Design review of the part built by this model. Coordinates are the model's own, in mm. Face numbers are marked on the shaded views. Coordinates: 2 decimals unless noted, no trailing zeros. Write each loop counter-clockwise with the first axis right and the second up, starting at its lowest first coordinate (ties: lowest second). Pieces come first, ordered by that corner, then holes. Notation, with made-up numbers: (-33, -4.5) - (10, -4.5) arc R17 ccw to (10, 11.5) - close; hole circle Ø6 at (48, -32.75). An arc over 180 degrees is marked (long way). Answer as a JSON object with one key per item and string values.
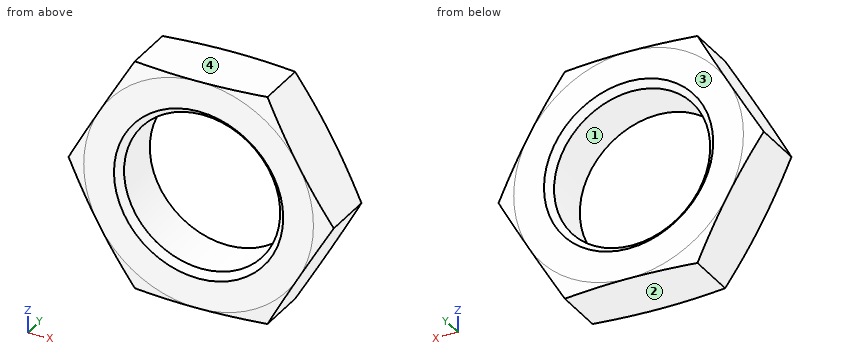
```python
from build123d import *

# Parameters (mm, degrees)
CUT_EXTRUDE1_DEPTH      = 2.5
CUT_EXTRUDE1_DEPTH_BACK = 2.5
SKETCH2_R               = 20


with BuildPart() as part:
    # Sketch1 → Revolve1 (revolve)
    with BuildSketch(Plane.XY, mode=Mode.PRIVATE) as revolve1_sk:
        Polygon((6.4585, -1.9585), (7, -2.5), (9.5, -2.5), (15, -1.026279442), (15, 1.026279442), (9.5, 2.5), (7, 2.5), (6.4585, 1.9585), align=None)
    revolve(revolve1_sk.sketch.rotate(Axis((0, -2.5, 0), (0, 1, 0)), 270), axis=Axis((0, -2.5, 0), (0, 1, 0)))

    # Sketch2 → Cut-Extrude1 (cut, two sides: drawn at the far end of the back side and taken through both)
    with BuildSketch(Plane(origin=(0, 0, 0), x_dir=(1, 0, 0), z_dir=(0, 1, 0)).offset(-CUT_EXTRUDE1_DEPTH_BACK)):
        Circle(SKETCH2_R)
        Polygon((-10.969655115, 0), (-5.484827557, -9.5), (5.484827557, -9.5), (10.969655115, 0), (5.484827557, 9.5), (-5.484827557, 9.5), align=None, mode=Mode.SUBTRACT)
    extrude(amount=CUT_EXTRUDE1_DEPTH + CUT_EXTRUDE1_DEPTH_BACK, mode=Mode.SUBTRACT)


solid = part.part
```
(1) To check wall thickness, follow line 1 (Z direction, x = -4.75, y = 1.4); line 2 (X direction, y = -0.45, z = -0.5); line 3 (X direction, y = -2, z = 0.25). State the ranges of each line that lie inside material, in increasing order. Write a range as from..to.
Solved:
{"line 1": "z = -9.5..-4.38, 4.38..9.5", "line 2": "x = -10.68..-6.44, 6.44..10.68", "line 3": "x = -10.83..-6.5, 6.5..10.83"}
(2) Take a section at A-A, the plane y = -1.2. Write out the cut boundary in (x, z).
Solved:
{"outline": "(-10.97, 0) - (-5.48, -9.5) - (5.48, -9.5) - (10.97, 0) - (5.48, 9.5) - (-5.48, 9.5) - close; hole circle Ø12.92 at (0, 0)"}
(3) The part is to be moulded in two halves that separate along Z. For the marked faces 1, 2, 3 and 4, say which applies: pulls with the +Z half, pulls with the -Z half, needs draft (parallel to the pull), parting line crosses it, or undercut.
Solved:
{"face 1": "undercut", "face 2": "pulls with the -Z half", "face 3": "needs draft", "face 4": "pulls with the +Z half"}
